Could you check a few things on this drawing? It's one solid part, dimensions in mm from its lowest x, y, z. A direction names the side the tool comes from. Round coordinates to 2 decimals unless told otherwise and drop trailing zeros. Order: outer loops, then holes, each group sorted by start corner. A loop starts at its lowest first (then second) coordinate and runs counter-clockwise, first axis right, second up. Notation, with made-up numbers: (63, 27.25) - (97, 27.25) arc R14 ccw to (97, 52.25) - close; hole circle Ø2 at (56.25, 44.25). An arc over 180 degrees is marked (long way). Use one line per item in the form item = value.
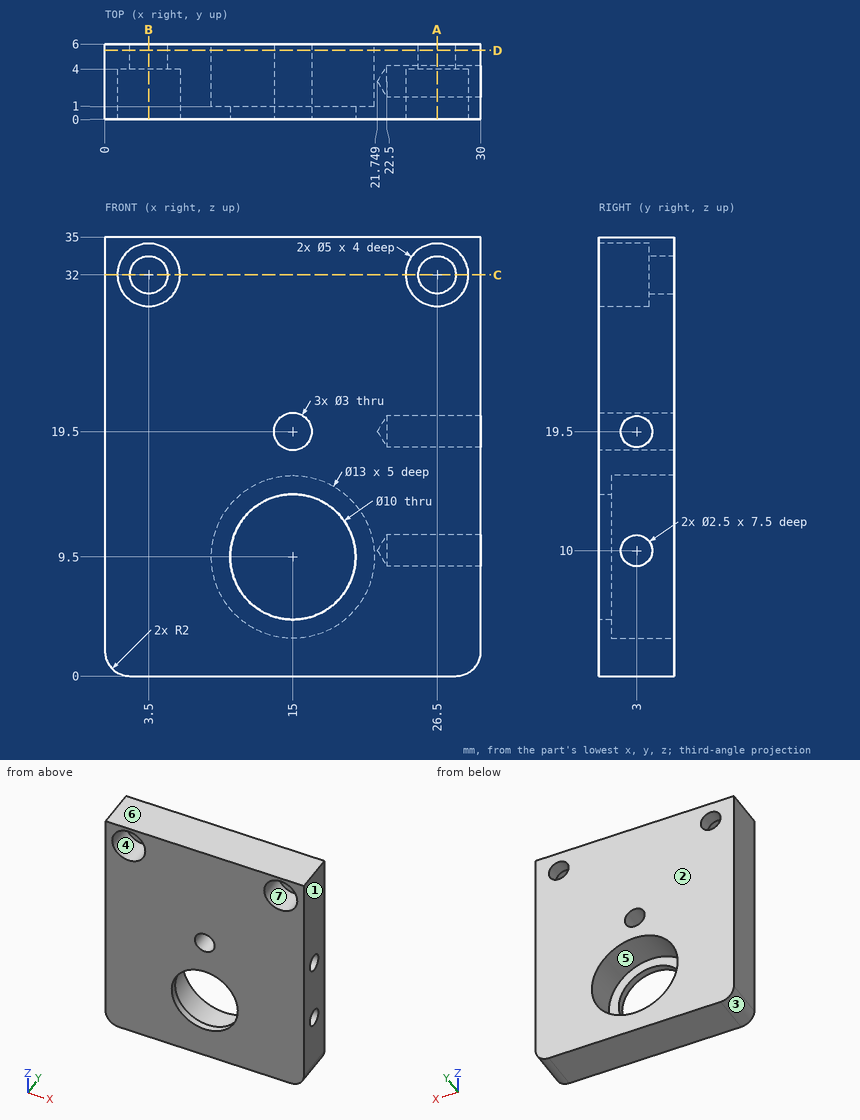
Item 1: If we mould it in two halves opening along X, with no side actions, what happens to the marked faces 1, 2, 3 and 4? For each: released by +X, released by -X, zero draft, split by the parting line, or undercut.
Found:
face_1 = released by +X
face_2 = zero draft
face_3 = released by -X
face_4 = undercut
Item 2: Will these pins go through, and if not, where does the flat tip stop? P1, Ø2, axis at y = 3, z = 10, coming from the +X side; P2, Ø1.5, axis at x = 13, z = 7.5, coming from the +Y side; P3, Ø11.5, axis at x = 15, z = 9.5, coming from the +Y side; P4, Ø1.5, axis at y = 3, z = 19.5, coming from the +X side.
Found:
P1 = 22.35
P2 = through
P3 = 1
P4 = 22.2
Item 3: Imagine slicing it at A-A on x = 26.5. Please give me the cut outline in (y, z).
Found:
outline = (0, 0) - (6, 0) - (6, 30.5) - (4, 30.5) - (4, 29.5) - (0, 29.5) - close; (0, 34.5) - (4, 34.5) - (4, 33.5) - (6, 33.5) - (6, 35) - (0, 35) - close; hole circle Ø2.5 at (3, 10); hole circle Ø2.5 at (3, 19.5)
Item 4: Imagine slicing it at D-D on y = 5.5. Please give me the cut outline in (x, z), plus the area to 3 significant figures.
Found:
outline = (0, 2) arc R2 ccw to (2, 0) - (28, 0) arc R2 ccw to (30, 2) - (30, 35) - (0, 35) - close; hole circle Ø3 at (3.5, 32); hole circle Ø13 at (15, 9.5); hole circle Ø3 at (15, 19.5); hole circle Ø3 at (26.5, 32)
area = 894 mm2
Item 5: Imagine slicing it at C-C on z = 32. Please give me the cut outline in (x, y), plus the area to 3 significant figures.
Found:
outline = (0, 0) - (1, 0) - (1, 4) - (2, 4) - (2, 6) - (0, 6) - close; (5, 4) - (6, 4) - (6, 0) - (24, 0) - (24, 4) - (25, 4) - (25, 6) - (5, 6) - close; (28, 4) - (29, 4) - (29, 0) - (30, 0) - (30, 6) - (28, 6) - close
area = 128 mm2
Item 6: For the marked faces 5, 6 and 7, which set-ups out of +Z, -Z, +X, -X, +Y, -Y let a thin tool reach every point of the face, with its end or its side?
Found:
face_5 = +Y
face_6 = +Z, +X, -X, +Y, -Y
face_7 = -Y
Item 7: Imagine slicing it at B-B on x = 3.5. Please give me the cut outline in (y, z), plus the area to 3 significant figures.
Found:
outline = (0, 0) - (6, 0) - (6, 30.5) - (4, 30.5) - (4, 29.5) - (0, 29.5) - close; (0, 34.5) - (4, 34.5) - (4, 33.5) - (6, 33.5) - (6, 35) - (0, 35) - close
area = 184 mm2
Item 8: I need wall thicknesses on L1, parallel to X at y = 5.45, z = 32; L2, parallel to Z at x = 26, y = 3; L3, parallel to Y at x = 27, z = 19.5. Which ranges of each line are inside material? Lowest first, please.
Found:
L1 = 0 to 2, 5 to 25, 28 to 30
L2 = 0 to 8.75, 11.25 to 18.25, 20.75 to 29.55, 34.45 to 35
L3 = 0 to 1.75, 4.25 to 6
